Source: CAD feature listing. Evaluate the final solid. Frame: model axes, mm. Face numbers are marked on the shaded views. A direction names the side the tool comes from. Coordinates: 2 decimals unless noted, no trailing zeros. Order: outer loops, then holes, each group sorted by start corner. A loop starts at its lowest first (then second) coordinate and runs counter-clockwise, first axis right, second up. Notation, with made-up numbers: (39.25, 77.25) -> (52.25, 77.25) arc R17 cw to (52.25, 107.25) -> close; hole circle Ø5 at (29.5, -20.75). An arc over 180 degrees is marked (long way). Write item = value, one per line. Start each with the question number.
Item 1: Section query B-B (x = -11.5). Output: boundary loops of the cut face in (y, z), then the cut area to 3 significant figures.
Item 2: Section query D-D (z = -1.5). Output: boundary loops of the cut face in (x, y).
Item 3: Section query A-A (y = 74.5). Output: boundary loops of the cut face in (x, z), then the cut area to 3 significant figures.
Item 4: Contact query for flat-ended pins moving along their axis: pin 1 (3 mm diameter, centred on x = 6.5, z = -12.5, fed in from +Y); pin 2 (6 mm diameter, centred on x = -11.5, y = 9, fed in from +Z); pin 3 (11 mm diameter, centred on x = -8, y = 43.5, fed in from -Z); pin 4 (11.5 mm diameter, centred on x = 11.5, y = 9, fed in from +Z). Output: stop coordinate, or through.
Item 5: Section query C-C (z = -9.5). Output: boundary loops of the cut face in (x, y), then the cut area to 3 significant figures.
Item 6: Set-up query: the marked faces 1, 2 and 3. Return all of +Z, -Z, +X, -X, +Y, -Y with unobstructed straight access to the full face (end or side cutting, diameter ignored); none if empty.
Item 7: Mould query, pull axis X, two halves, no side actions, for the marked faces 4, 5, 6 and 7. Classes: released by +X, released by -X, zero draft, split by the parting line, or undercut.
Item 8: Ray query, line 1 along Y through (x, z) = (-11.5, -5.5); line 2 along Z through (x, y) = (-2.5, 69); line 3 along Y through (x, z) = (15, -3.75). Return the intervals inside material, ascending. Write a range as [from, to].
```python
from build123d import *

# Parameters (mm, degrees)
BOSS_EXTRUDE1_DEPTH                                  = 18
HOLE_SIZE_PER_SOCKET_HEAD_CAP_SCREW_TYPE_D           = 5.5
HOLE_SIZE_PER_SOCKET_HEAD_CAP_SCREW_TYPE_CBORE_D     = 10
HOLE_SIZE_PER_SOCKET_HEAD_CAP_SCREW_TYPE_CBORE_DEPTH = 5.7
SKETCH5_R                                            = 3
CUT_EXTRUDE1_DEPTH                                   = 86.111691324
CHAMFER1_SIZE                                        = 1
CUT_EXTRUDE3_DEPTH                                   = 0.5


with BuildPart() as part:
    # Sketch1 → Boss-Extrude1 (new, symmetric)
    with BuildSketch(Plane(origin=(0, 0, 0), x_dir=(0, 0, -1), z_dir=(1, 0, 0))):
        Polygon((14, 0), (0, 0), (0, 82), (8, 82), (8, 18), (14, 18), align=None)
    extrude(amount=BOSS_EXTRUDE1_DEPTH, both=True)

    # Hole size per socket head cap screw type1 (through all)
    with Locations(Plane.XY):
        with Locations((11.5, 9), (-11.5, 9)):
            CounterBoreHole(HOLE_SIZE_PER_SOCKET_HEAD_CAP_SCREW_TYPE_D / 2, HOLE_SIZE_PER_SOCKET_HEAD_CAP_SCREW_TYPE_CBORE_D / 2, HOLE_SIZE_PER_SOCKET_HEAD_CAP_SCREW_TYPE_CBORE_DEPTH)

    # Sketch5 → Cut-Extrude1 (cut, through all)
    with BuildSketch(Plane.XY):
        with Locations((-11.5, 74.5)):
            Circle(SKETCH5_R)
        with Locations(Location((11.5, 74.5, 0), (0, 0, 270))):
            Circle(SKETCH5_R)
    extrude(amount=-CUT_EXTRUDE1_DEPTH, mode=Mode.SUBTRACT)

    # Chamfer1
    chamfer1_edges = [part.edges().sort_by_distance(p)[0] for p in [
        (18, 82, -4),
        (18, 0, -7),
        (-18, 0, -7),
        (-18, 82, -4),
    ]]
    chamfer(chamfer1_edges, length=CHAMFER1_SIZE)

    # Sketch6 → Cut-Extrude3 (cut)
    with BuildSketch(Plane.XY):
        Polygon((6.7, 44), (17.896152423, 41), (6.7, 38), align=None)
    extrude(amount=-CUT_EXTRUDE3_DEPTH, mode=Mode.SUBTRACT)


solid = part.part
```
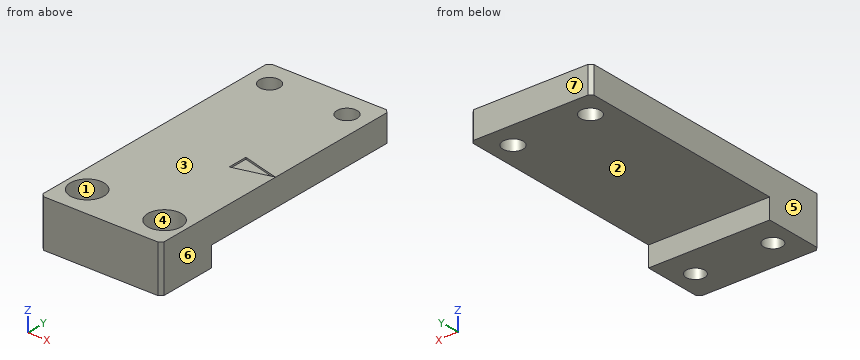
Computed:
q1.outline = (0, -14) -> (6.25, -14) -> (6.25, -5.7) -> (4, -5.7) -> (4, 0) -> (0, 0) -> close; (11.75, -14) -> (18, -14) -> (18, -8) -> (71.5, -8) -> (71.5, 0) -> (14, 0) -> (14, -5.7) -> (11.75, -5.7) -> close; (77.5, -8) -> (82, -8) -> (82, 0) -> (77.5, 0) -> close
q1.area = 613 mm^2
q2.outline = (-18, 1) -> (-17, 0) -> (17, 0) -> (18, 1) -> (18, 81) -> (17, 82) -> (-17, 82) -> (-18, 81) -> close; hole circle Ø10 at (-11.5, 9); hole circle Ø6 at (-11.5, 74.5); hole circle Ø10 at (11.5, 9); hole circle Ø6 at (11.5, 74.5)
q3.outline = (-18, -8) -> (-14.5, -8) -> (-14.5, 0) -> (-18, 0) -> close; (-8.5, -8) -> (8.5, -8) -> (8.5, 0) -> (-8.5, 0) -> close; (14.5, -8) -> (18, -8) -> (18, 0) -> (14.5, 0) -> close
q3.area = 192 mm^2
q4.pin_1 = 18
q4.pin_2 = -5.7
q4.pin_3 = -8
q4.pin_4 = 0
q5.outline = (-18, 1) -> (-17, 0) -> (17, 0) -> (18, 1) -> (18, 18) -> (-18, 18) -> close; hole circle Ø5.5 at (-11.5, 9); hole circle Ø5.5 at (11.5, 9)
q5.area = 599 mm^2
q6.face_1 = +Z
q6.face_2 = -Z, +X, -X, +Y
q6.face_3 = +Z, +X, -X, +Y, -Y
q7.face_4 = undercut
q7.face_5 = released by -X
q7.face_6 = released by +X
q7.face_7 = zero draft
q8.line_1 = [0, 4], [14, 71.5], [77.5, 82]
q8.line_2 = [-8, 0]
q8.line_3 = [0, 5.43], [12.57, 82]
